Study the drawing (mm; zero at the part's minimum x, y, z) and answer. Coordinates: 2 decimals unless noted, no trailing zeros. Order: outer loops, then holes, each group sorted by start corner. A loop starts at its lowest first (then second) coordinate and runs counter-clockwise, first axis right, second up. Notation, with made-up numbers: M 61.5,-20.5 L 66.5,-20.5 A19 cw 66.5,3.5 Z; hole C 4.25,39.25 d11. An arc over 180 degrees is marked long. One line per item, written item: value. Start each with the question number.
Q1. The part is cut by section C-C on z = 4. Give the vertices of the cut face in (x, y), then the cut area to 3 significant figures.
Q2. Each of these flat-tipped pins is pushed along its axis until it touches: pin 1 Ø5 at (y, z) = (3.5, 18) entering from -X; pin 2 Ø4.5 at (x, y) = (12.5, 10) entering from +Z. Where does it stop, or does it pass through?
Q3. Straight lines are drawn through the part: line 1 along Y through (x, z) = (42.5, 13); line 2 along X through (y, z) = (10.75, 6.5); line 3 along X through (y, z) = (7.75, 8.25). For each, find the intervals that lie inside material, in ascending order. Write a range as [from, to].
Q4. The part is cut by section A-A on x = 42.5. Give the vertices of the cut face in (y, z), then the cut area to 3 significant figures.
Q5. The part is cut by section B-B on y = 10. Give the vertices of the cut face in (x, z), then the cut area to 3 significant figures.
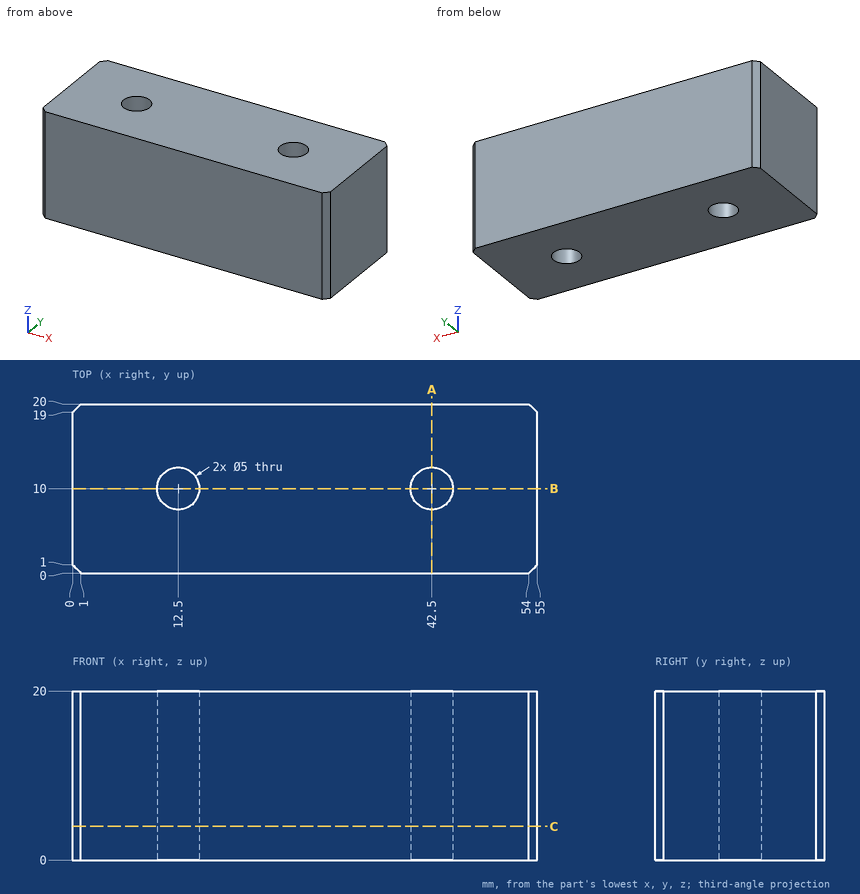
Output:
1. outline: M 0,1 L 1,0 L 54,0 L 55,1 L 55,19 L 54,20 L 1,20 L 0,19 Z; hole C 12.5,10 d5; hole C 42.5,10 d5
1. area: 1,060 mm^2
2. pin 1: stops at x = 0
2. pin 2: passes through
3. line 1: y = [0, 7.5], [12.5, 20]
3. line 2: x = [0, 10.12], [14.88, 40.12], [44.88, 55]
3. line 3: x = [0, 11.41], [13.59, 41.41], [43.59, 55]
4. outline: M 0,0 L 7.5,0 L 7.5,20 L 0,20 Z; M 12.5,0 L 20,0 L 20,20 L 12.5,20 Z
4. area: 300 mm^2
5. outline: M 0,0 L 10,0 L 10,20 L 0,20 Z; M 15,0 L 40,0 L 40,20 L 15,20 Z; M 45,0 L 55,0 L 55,20 L 45,20 Z
5. area: 900 mm^2
